```python
from build123d import *
from build123d.topology import SkipClean

# Parameters (mm, degrees)
SKETCH1_R           = 5
BOSS_EXTRUDE1_DEPTH = 220
CHAMFER1_SIZE       = 0.5
CUT_EXTRUDE1_DEPTH  = 12


with BuildPart() as part:
    # Sketch1 → Boss-Extrude1 (new body)
    with BuildSketch(Plane(origin=(0, 0, 0), x_dir=(1, 0, 0), z_dir=(0, 1, 0))):
        with Locations(Location((0, 0, 0), (0, 0, 270))):
            Circle(SKETCH1_R)
    extrude(amount=BOSS_EXTRUDE1_DEPTH)

    # Chamfer1
    chamfer1_edges = [part.edges().sort_by_distance(p)[0] for p in [
        (0, 0, -5),
        (0, 220, -5),
    ]]
    chamfer(chamfer1_edges, length=CHAMFER1_SIZE)

    # Sketch2 → Cut-Extrude1 (cut)
    with SkipClean():  # the faces are left unmerged after this step: merging them gives an invalid solid
        with BuildSketch(Plane(origin=(0, 0, 0), x_dir=(1, 0, 0), z_dir=(0, 1, 0))):
            with BuildLine():
                Line((-2.179449472, 4.5), (2.179449472, 4.5))
                ThreePointArc((2.179449472, 4.5), (0, 5), (-2.179449472, 4.5))
            make_face()
        extrude(amount=CUT_EXTRUDE1_DEPTH, mode=Mode.SUBTRACT)


solid = part.part
```
Verification items for the finished model (mm, model axes). A direction names the side the tool comes from. Round coordinates to 2 decimals unless told otherwise and drop trailing zeros. Order: outer loops, then holes, each group sorted by start corner. A loop starts at its lowest first (then second) coordinate and runs counter-clockwise, first axis right, second up. Notation, with made-up numbers: (-23, 61) -> (18, 61) arc R19 ccw to (18, 72) -> close; hole circle Ø11 at (24.5, 46.5). An arc over 180 degrees is marked (long way). Put each result on its own line as item: value. Start each with the question number.
(1) Section check A-A (y = 89). Enter the section's corners in (x, z), then the cut area to 3 significant figures.
(2) Tool access check on faces 1 (the face through (0, 6, -4.5)), 2 (the face through (0, 220, 0)). Record the directions out of +Z, -Z, +X, -X, +Y, -Y that give a thin tool (end or side, any length) a straight path to the whole face; none if there is none.
(3) Depth check by flat-ended pin: pin 1 Ø4 at (y, z) = (70.5, 2) entering from -X; pin 2 Ø2 at (y, z) = (114, 2) entering from -X; pin 3 Ø2 at (x, y) = (0.5, 4.5) entering from -Z; pin 4 Ø1.5 at (y, z) = (152.5, 2) entering from +X. Enter the tip coordinate at first touch or a pass-through.
(4) Material ranges on line 1 along Z through (x, y) = (-4.5, 146); line 2 along Z through (x, y) = (0.5, 175.5); line 3 along Y through (x, z) = (-3.5, -3.25), recorded low to high.
Completed:
1. outline: circle Ø10 at (0, 0)
1. area: 78.5 mm2
2. face 1: -Z, +X, -X, -Y
2. face 2: +Z, -Z, +X, -X, +Y
3. pin 1: stops at x = -5
3. pin 2: stops at x = -4.9
3. pin 3: stops at z = -4.5
3. pin 4: stops at x = 4.84
4. line 1: z = -2.18 to 2.18
4. line 2: z = -4.97 to 4.97
4. line 3: y = 0.28 to 219.72
